Part print with two shaded views. Sizes in mm from the minimum x, y, z corner. Round coordinates to 2 decimals unless told otherwise and drop trailing zeros. Loops run counter-clockwise (first coordinate to the right, second up) from the corner with the lowest first, then second, coordinate; pieces in that order, holes last. Notation, with made-up numbers: (53, 75.25) -> (79, 75.25) arc R25 ccw to (79, 92.25) -> close; hole circle Ø2 at (57.25, 29). An arc over 180 degrees is marked (long way). Use a Markdown table: item, result. Add a question column.
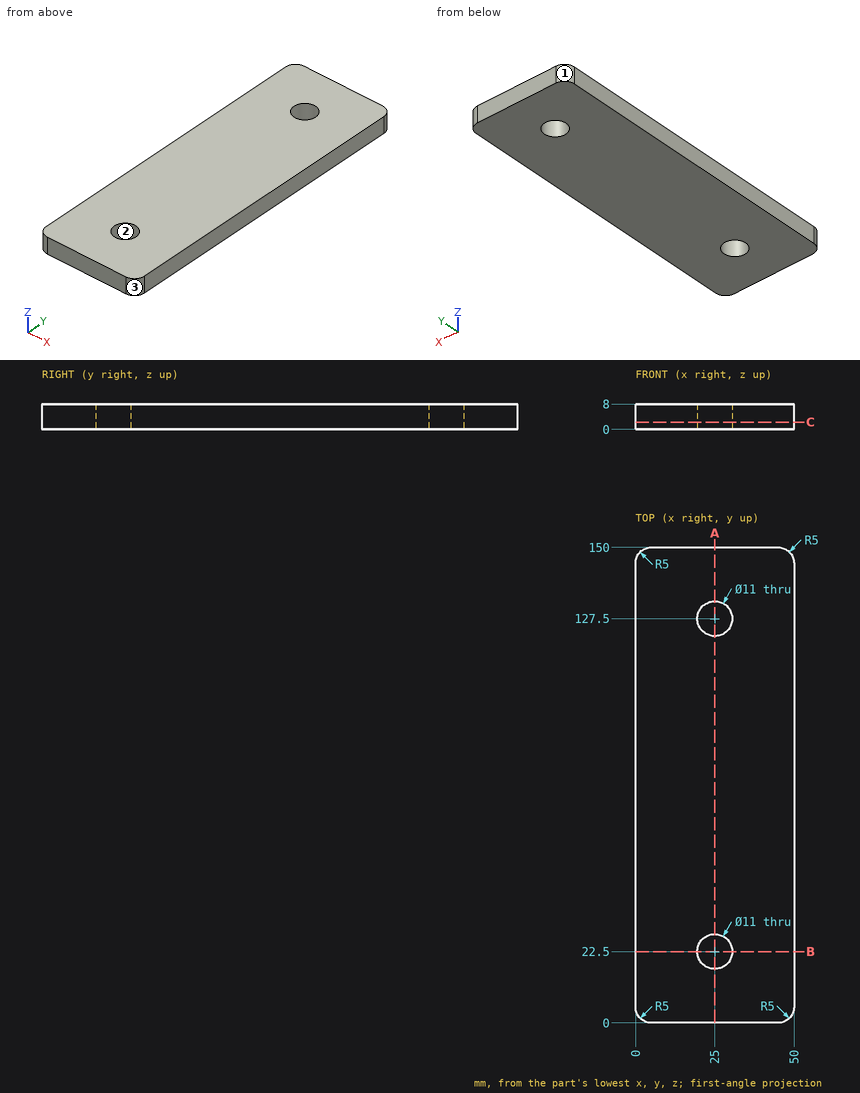
1) Cut at B-B on y = 22.5. Write the cut outline in (x, z), and give its area (3 significant figures).
2) Wall check: probe 1 along Y at (x, z) = (25, 5.25); probe 2 along X at (y, z) = (127, 6.75); probe 3 along Y at (x, z) = (20.5, 1). Give the ranges that are in metal, low to high. Write a range as from..to.
3) Cut at C-C on z = 2.25. Write the cut outline in (x, y), and give its area (3 significant figures).
4) Cut at A-A on x = 25. Write the cut outline in (y, z).
5) Pull direction X, two halves, no side cores. Call the marked faces 1, 2 and 3: +X half, -X half, draft (parallel to the pull), parting line (faces both ways), or undercut.
Established:
| question | item | result |
|---|---|---|
| 1 | outline | (0, 0) -> (19.5, 0) -> (19.5, 8) -> (0, 8) -> close; (30.5, 0) -> (50, 0) -> (50, 8) -> (30.5, 8) -> close |
| 1 | area | 312 mm^2 |
| 2 | probe 1 | y = 0..17, 28..122, 133..150 |
| 2 | probe 2 | x = 0..19.52, 30.48..50 |
| 2 | probe 3 | y = 0..19.34, 25.66..124.34, 130.66..150 |
| 3 | outline | (0, 5) arc R5 ccw to (5, 0) -> (45, 0) arc R5 ccw to (50, 5) -> (50, 145) arc R5 ccw to (45, 150) -> (5, 150) arc R5 ccw to (0, 145) -> close; hole circle Ø11 at (25, 22.5); hole circle Ø11 at (25, 127.5) |
| 3 | area | 7,290 mm^2 |
| 4 | outline | (0, 0) -> (17, 0) -> (17, 8) -> (0, 8) -> close; (28, 0) -> (122, 0) -> (122, 8) -> (28, 8) -> close; (133, 0) -> (150, 0) -> (150, 8) -> (133, 8) -> close |
| 5 | face 1 | -X half |
| 5 | face 2 | undercut |
| 5 | face 3 | +X half |
